Check sheet for the modelled part. Datum: model origin and axes. Units: mm. Face numbers are marked on the shaded views. A direction names the side the tool comes from. Round coordinates to 2 decimals unless told otherwise and drop trailing zeros. Order: outer loops, then holes, each group sorted by start corner. A loop starts at its lowest first (then second) coordinate and runs counter-clockwise, first axis right, second up.
(1) Sectioned sample at B-B, the plane y = 146.5. Enter the section's corners in (x, z).
(2) Sectioned sample at A-A, the plane x = -110. Enter the section's corners in (y, z), and give its area (3 significant figures).
(3) Tool access check on the marked faces 1, 2, 3, 4 and 5. Record the directions out of +Z, -Z, +X, -X, +Y, -Y that give a thin tool (end or side, any length) a straight path to the whole face; none if there is none.
(4) Sectioned sample at C-C, the plane x = 0. Enter the section's corners in (y, z).
(5) Thickness scan on probe 1 along Y at (x, z) = (-110, 11); probe 2 along X at (y, z) = (11.25, 0); probe 3 along X at (y, z) = (110, -11). Record the ranges inside material, lowest first.
(6) Sectioned sample at D-D, the plane x = 81. Enter the section's corners in (y, z), and give its area (3 significant figures).
(7) Depth check by flat-ended pin: pin 1 (17 mm diameter, centred on y = 162.5, z = 10.5, fed in from -X); pin 2 (2 mm diameter, centred on x = 14, z = 13.5, fed in from -Y); pin 3 (2 mm diameter, centred on x = -83.5, z = -12.5, fed in from +Y). Enter the tip coordinate at first touch or a pass-through.
```python
from build123d import *

# Parameters (mm, degrees)
BASE_BLOCK_DEPTH             = 40
LOWER_HUB_40_DEPTH           = 5
LOWER_HUB_40_DEPTH_BACK      = 65
LOWER_HUB_40_SKETCH_R        = 20
UPPER_HUB_56_SKETCH_R        = 28
UPPER_HUB_56_DEPTH           = 60
WEB_ARM_DEPTH                = 28
SPLIT_START                  = -101
SPLIT_SLOT_DEPTH             = 101
CLAMP_EAR_DEPTH              = 15
UPPER_BORE_20_SKETCH_R       = 10
UPPER_BORE_20_DEPTH          = 89
CLAMP_SCREW_HOLE_15_SKETCH_R = 7.5
CLAMP_SCREW_HOLE_15_DEPTH    = 89
LOWER_BORE_20_SKETCH_R       = 10
LOWER_BORE_20_DEPTH          = 89
MOUNTING_FOOT_DEPTH          = 20
FOOT_HOLE_16_SKETCH_R        = 8
FOOT_HOLE_16_DEPTH           = 45


with BuildPart() as part:
    # Base Block Sketch → Base Block (new, symmetric)
    with BuildSketch(Plane.XY):
        with BuildLine():
            Line((-60, 0), (-50, 0))
            ThreePointArc((-50, 0), (0, 50), (50, 0))
            Line((50, 0), (60, 0))
            ThreePointArc((60, 0), (0, 60), (-60, 0))
        make_face()
    extrude(amount=BASE_BLOCK_DEPTH, both=True)



with BuildPart() as body_2:
    # Lower Hub Ø40 Sketch → Lower Hub Ø40 (new, two sides: drawn at the far end of the back side and taken through both)
    with BuildSketch(Plane.XY.offset(28).offset(-LOWER_HUB_40_DEPTH_BACK)):
        with Locations((-110, 0)):
            Circle(LOWER_HUB_40_SKETCH_R)
    extrude(amount=LOWER_HUB_40_DEPTH + LOWER_HUB_40_DEPTH_BACK)


with BuildPart() as body_3:
    # Upper Hub Ø56 Sketch → Upper Hub Ø56 (new body)
    with BuildSketch(Plane(origin=(-15, 0, 0), x_dir=(0, 0, -1), z_dir=(1, 0, 0))):
        with Locations((0, 150)):
            Circle(UPPER_HUB_56_SKETCH_R)
    extrude(amount=-UPPER_HUB_56_DEPTH)


with BuildPart() as part_1:
    add(part.part)

    add(body_2.part)  # Web Arm merges body 2

    add(body_3.part)  # Web Arm merges body 3
    # Web Arm Profile → Web Arm (add, symmetric)
    with BuildSketch(Plane.XY):
        with BuildLine():
            Line((-55, 74.446056073), (-55, 150))
            Line((-55, 150), (-65, 150))
            Line((-65, 150), (-65, 40.311288741))
            ThreePointArc((-65, 40.311288741), (-76.823843083, 19.065374102), (-101.111111111, 17.91612833))
            ThreePointArc((-101.111111111, 17.91612833), (-93.003268288, 10.540925534), (-90, 0))
            Line((-90, 0), (-60, 0))
            ThreePointArc((-60, 0), (-39.037382491, 45.564051271), (9.202758941, 59.290043244))
            ThreePointArc((9.202758941, 59.290043244), (-15.279998201, 72.92654907), (-25, 99.211169164))
            Line((-25, 99.211169164), (-25, 150))
            Line((-25, 150), (-35, 150))
            Line((-35, 150), (-35, 99.211169164))
            ThreePointArc((-35, 99.211169164), (-34.000437544, 89.223422766), (-31.041398663, 79.631848749))
            ThreePointArc((-31.041398663, 79.631848749), (-31.260550889, 71.378609178), (-37.611325277, 66.103037571))
            Line((-37.611325277, 66.103037571), (-42.35537658, 64.802095944))
            ThreePointArc((-42.35537658, 64.802095944), (-51.064394685, 66.494759506), (-55, 74.446056073))
        make_face()
    extrude(amount=WEB_ARM_DEPTH, both=True)

    # Split Slot Sketch → Split Slot (cut)
    with BuildSketch(Plane.ZY.offset(75).offset(SPLIT_START)):
        with BuildLine():
            Line((-2.5, 150), (0, 150))
            Line((0, 150), (2.5, 150))
            Line((2.5, 150), (2.5, 159.682458366))
            Line((2.5, 159.682458366), (2.5, 177.888169535))
            ThreePointArc((2.5, 177.888169535), (0, 178), (-2.5, 177.888169535))
            Line((-2.5, 177.888169535), (-2.5, 159.682458366))
            Line((-2.5, 159.682458366), (-2.5, 150))
        make_face()
        with BuildLine():
            Line((2.5, 150), (0, 150))
            Line((0, 150), (-2.5, 150))
            Line((-2.5, 150), (-2.5, 159.682458366))
            ThreePointArc((-2.5, 159.682458366), (0, 140), (2.5, 159.682458366))
            Line((2.5, 159.682458366), (2.5, 150))
        make_face()
    extrude(amount=SPLIT_SLOT_DEPTH, mode=Mode.SUBTRACT)

    # Clamp Ear Sketch → Clamp Ear (add)
    with BuildSketch(Plane.XY.offset(-2.5)):
        with BuildLine():
            Line((-31.323438353, 177.888169535), (-31.323438353, 149.888169535))
            Line((-31.323438353, 149.888169535), (-61.323438353, 150))
            Line((-61.323438353, 150), (-61.323438353, 177.888169535))
            Line((-61.323438353, 177.888169535), (-61.323438353, 189.888169535))
            ThreePointArc((-61.323438353, 189.888169535), (-46.323438353, 204.888169535), (-31.323438353, 189.888169535))
            Line((-31.323438353, 189.888169535), (-31.323438353, 177.888169535))
        make_face()
    clamp_ear = extrude(amount=-CLAMP_EAR_DEPTH)

    # Clamp Ear Mirror: Clamp Ear across plane
    add(clamp_ear.mirror(Plane.XY))

    # Upper Bore Ø20 Sketch → Upper Bore Ø20 (cut)
    with BuildSketch(Plane(origin=(-15, 0, 0), x_dir=(0, 0, -1), z_dir=(1, 0, 0))):
        with Locations((0, 150)):
            Circle(UPPER_BORE_20_SKETCH_R)
    extrude(amount=-UPPER_BORE_20_DEPTH, mode=Mode.SUBTRACT)

    # Clamp Screw Hole Ø15 Sketch → Clamp Screw Hole Ø15 (cut)
    with BuildSketch(Plane.XY.offset(17.5)):
        with Locations((-46.323438353, 189.888169535)):
            Circle(CLAMP_SCREW_HOLE_15_SKETCH_R)
    extrude(amount=-CLAMP_SCREW_HOLE_15_DEPTH, mode=Mode.SUBTRACT)

    # Lower Bore Ø20 Sketch → Lower Bore Ø20 (cut)
    with BuildSketch(Plane.XY.offset(33)):
        with Locations((-110, 0)):
            Circle(LOWER_BORE_20_SKETCH_R)
    extrude(amount=-LOWER_BORE_20_DEPTH, mode=Mode.SUBTRACT)

    # Mounting Foot Sketch → Mounting Foot (add)
    with BuildSketch(Plane.XZ):
        with BuildLine():
            Line((100, 0), (100, 15))
            ThreePointArc((100, 15), (97.071067812, 22.071067812), (90, 25))
            Line((90, 25), (50, 25))
            Line((50, 25), (50, -25))
            Line((50, -25), (90, -25))
            ThreePointArc((90, -25), (97.071067812, -22.071067812), (100, -15))
            Line((100, -15), (100, 0))
        make_face()
    extrude(amount=-MOUNTING_FOOT_DEPTH)

    # Foot Hole Ø16 Sketch → Foot Hole Ø16 (cut)
    with BuildSketch(Plane(origin=(0, 20, 0), x_dir=(1, 0, 0), z_dir=(0, 1, 0))):
        with Locations(Location((78.284271247, 0, 0), (0, 0, 270))):
            Circle(FOOT_HOLE_16_SKETCH_R)
    extrude(amount=-FOOT_HOLE_16_DEPTH, mode=Mode.SUBTRACT)


solid = part_1.part
```
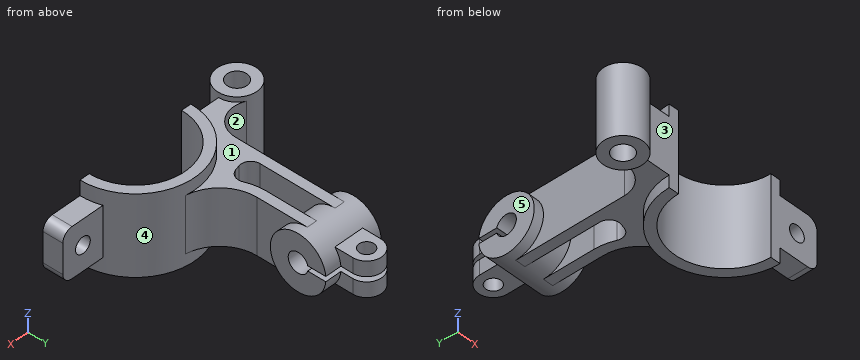
Derived:
1. outline: (-75, -27.78) - (-65, -27.78) - (-65, -28) - (-55, -28) - (-55, -27.78) - (-35, -27.78) - (-35, -28) - (-25, -28) - (-25, -27.78) - (-15, -27.78) - (-15, -9.37) - (-75, -9.37) - close; (-75, 9.37) - (-15, 9.37) - (-15, 27.78) - (-25, 27.78) - (-25, 28) - (-35, 28) - (-35, 27.78) - (-55, 27.78) - (-55, 28) - (-65, 28) - (-65, 27.78) - (-75, 27.78) - close
2. outline: (-20, -37) - (-10, -37) - (-10, 33) - (-20, 33) - close; (10, -37) - (20, -37) - (20, 33) - (10, 33) - close
2. area: 1,400 mm2
3. face 1: +Z, +Y
3. face 2: +Z, -Z
3. face 3: +Z, -Z, +X, -Y
3. face 4: +Y
3. face 5: +Z, -Z, -X, +Y
4. outline: (50, -40) - (60, -40) - (60, -28) - (61.86, -28) - (61.86, 28) - (60, 28) - (60, 40) - (50, 40) - close
5. probe 1: y = -20 to -10, 10 to 20
5. probe 2: x = -126.54 to -48.72, 48.72 to 70.28, 86.28 to 100
5. probe 3: x = -65 to -55, -35 to -25
6. outline: (0, -25) - (20, -25) - (20, -7.52) - (0, -7.52) - close; (0, 7.52) - (20, 7.52) - (20, 25) - (0, 25) - close
6. area: 699 mm2
7. pin 1: stops at x = -75
7. pin 2: stops at y = 47.7
7. pin 3: stops at y = 16.46
